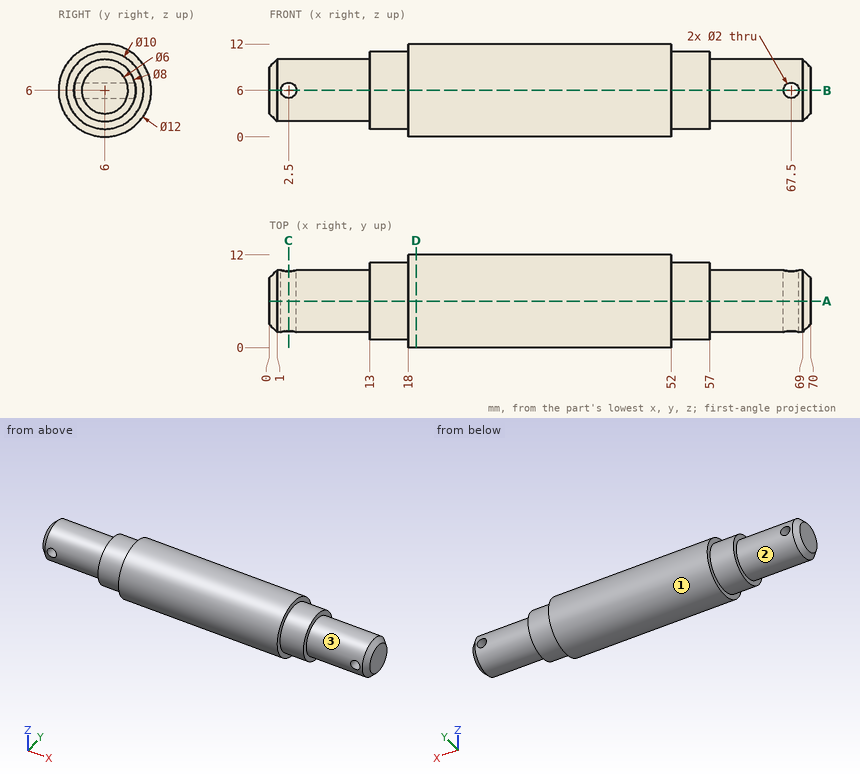
Study the drawing (mm; zero at the part's minimum x, y, z) and answer. A direction names the side the tool comes from. Coordinates: 2 decimals unless noted, no trailing zeros. Write each loop counter-clockwise with the first axis right and the second up, starting at its lowest first coordinate (ties: lowest second). Pieces come first, ordered by that corner, then holes. Notation, with made-up numbers: (46, -32.5) - (57, -32.5) arc R14 cw to (57, -21.5) - close; hole circle Ø10 at (-29, -35). An arc over 180 degrees is marked (long way). One line per item, written item: value.
1) Each of these flat-tipped pins is pushed along its axis until it touches: pin 1 Ø4 at (x, z) = (54.5, 11) entering from +Y; pin 2 Ø3 at (x, z) = (32, 9) entering from +Y; pin 3 Ø4 at (x, y) = (55, 2) entering from +Z; pin 4 Ø3.5 at (y, z) = (9, 8.5) entering from -X. Where does it stop, or does it pass through?
Geometry check:
pin 1: stops at y = 10
pin 2: stops at y = 11.81
pin 3: stops at z = 10.58
pin 4: stops at x = 0
2) Find section B-B (z = 6). Count the separate pieces of the cut face and the enclosed holes in it, and give its area (3 significant figures).
Geometry check:
separate pieces: 3
enclosed holes: 0
area: 682 mm2
3) Consider line 1 along X through (y, z) = (6.75, 6); line 2 along Z through (x, y) = (67.5, 8); line 3 along X through (y, z) = (2.25, 3.5). Determine where each line is inside the solid, lowest interval first. Write a range as from..to.
Geometry check:
line 1: x = 0..1.5, 3.5..66.5, 68.5..70
line 2: z = 2.54..5, 7..9.46
line 3: x = 13..57
4) Find section C-C (x = 2.5). Give the vertices of the cut face in (y, z), and give its area (3 significant figures).
Geometry check:
outline: (2.13, 5) arc R4 ccw to (9.87, 5) - close; (2.13, 7) - (9.87, 7) arc R4 ccw to start
area: 34.4 mm2
5) Find section D-D (x = 19). Give the vertices of the cut face in (y, z), and give its area (3 significant figures).
Geometry check:
outline: circle Ø12 at (6, 6)
area: 113 mm2
6) Find section A-A (y = 6). Give the vertices of the cut face in (x, z).
Geometry check:
outline: (0, 3) - (1, 2) - (13, 2) - (13, 1) - (18, 1) - (18, 0) - (52, 0) - (52, 1) - (57, 1) - (57, 2) - (69, 2) - (70, 3) - (70, 9) - (69, 10) - (57, 10) - (57, 11) - (52, 11) - (52, 12) - (18, 12) - (18, 11) - (13, 11) - (13, 10) - (1, 10) - (0, 9) - close; hole circle Ø2 at (2.5, 6); hole circle Ø2 at (67.5, 6)
7) A tool of negligible diameter and unlimited length cuts with its end or side. For the marked faces 1, 2 and 3, from which of +Z, -Z, +X, -X, +Y, -Y can it reach the whole face along a straight path? Write none if from no direction.
Geometry check:
face 1: +X, -X
face 2: -X
face 3: +X
